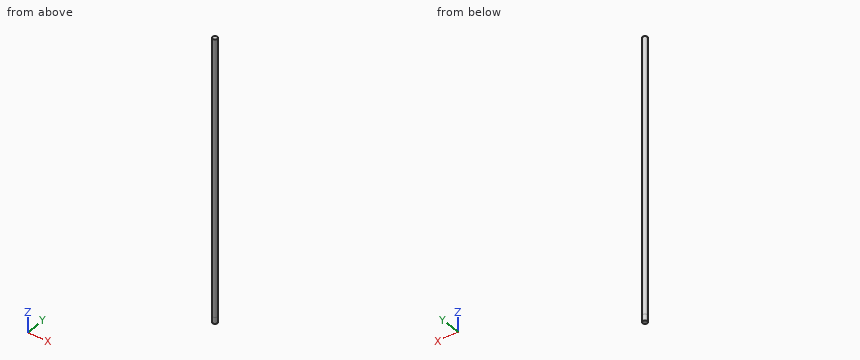
```python
from build123d import *

# Parameters (mm, degrees)
SKETCH_1_R          = 12.5
EXTRUDE_1_DEPTH     = 1470
EXTRUDE_START       = 50
SKETCH_9_R          = 12.5
EXTRUDE_5_DEPTH     = 50
SKETCH_2_W          = 0.55
SKETCH_2_H          = 1.3
CUT_EXTRUDE_START   = -16.5
SKETCH_11_R         = 12.5
CUT_EXTRUDE_2_DEPTH = 16.5
SKETCH_12_R         = 12.5
CUT_EXTRUDE_3_DEPTH = 16.5


with BuildPart() as part:
    # 草图1 → 凸台-拉伸1 (new body)
    with BuildSketch(Plane.XY):
        Circle(SKETCH_1_R)
    extrude(amount=EXTRUDE_1_DEPTH)

    # 草图9 → 凸台-拉伸5 (add)
    with BuildSketch(Plane(origin=(0, 0, 0), x_dir=(-1, 0, 0), z_dir=(0, 0, -1)).offset(EXTRUDE_START)):
        Circle(SKETCH_9_R)
    extrude(amount=-EXTRUDE_5_DEPTH)

    # 草图2 → 切除-旋转1 (revolve, cut)
    with BuildSketch(Plane(origin=(0, 0, 0), x_dir=(1, 0, 0), z_dir=(0, 1, 0)), mode=Mode.PRIVATE) as cut_revolve_1_sk:
        with Locations((12.225, -1450.65)):
            Rectangle(SKETCH_2_W, SKETCH_2_H)
        with Locations((-12.225, -1450.65)):
            Rectangle(SKETCH_2_W, SKETCH_2_H)
        with Locations((-12.225, 30.65)):
            Rectangle(SKETCH_2_W, SKETCH_2_H)
        with Locations((12.225, 30.65)):
            Rectangle(SKETCH_2_W, SKETCH_2_H)
    revolve(cut_revolve_1_sk.sketch.rotate(Axis((0, 0, 1476.033406801), (0, 0, 1)), 180), axis=Axis((0, 0, 1476.033406801), (0, 0, 1)), mode=Mode.SUBTRACT)

    # 草图11 → 切除-拉伸2 (cut)
    with BuildSketch(Plane.XY.offset(1470).offset(CUT_EXTRUDE_START)):
        with Locations(Location((0, 0, 0), (0, 0, 180))):
            Circle(SKETCH_11_R)
    extrude(amount=CUT_EXTRUDE_2_DEPTH, mode=Mode.SUBTRACT)

    # 草图12 → 切除-拉伸3 (cut)
    with BuildSketch(Plane(origin=(0, 0, -50), x_dir=(-1, 0, 0), z_dir=(0, 0, -1))):
        Circle(SKETCH_12_R)
    extrude(amount=-CUT_EXTRUDE_3_DEPTH, mode=Mode.SUBTRACT)


solid = part.part
```
Geometry: final body of the model. Coordinates: model frame, mm. Coordinates: 2 decimals unless noted, no trailing zeros. Order: outer loops, then holes, each group sorted by start corner. A loop starts at its lowest first (then second) coordinate and runs counter-clockwise, first axis right, second up. Notation, with made-up numbers: M 86,-5.75 L 131,-5.75 A29 cw 131,17.25 Z; hole C 79.5,9.5 d1. An arc over 180 degrees is marked long. Answer as CSV lines item,"result".
Q1. Section B-B on x = 6.25. Return the cut outline in (y, z), and give its area (3 significant figures).
Answers:
outline,"M -10.83,-33.5 L 10.83,-33.5 L 10.83,-31.3 L 10.19,-31.3 L 10.19,-30 L 10.83,-30 L 10.83,1450 L 10.19,1450 L 10.19,1451.3 L 10.83,1451.3 L 10.83,1453.5 L -10.83,1453.5 L -10.83,1451.3 L -10.19,1451.3 L -10.19,1450 L -10.83,1450 L -10.83,-30 L -10.19,-30 L -10.19,-31.3 L -10.83,-31.3 Z"
area,"32,200 mm^2"
Q2. Section A-A on y = -7.5. Return the cut outline in (x, z), and give its area (3 significant figures).
Answers:
outline,"M -10,-33.5 L 10,-33.5 L 10,-31.3 L 9.3,-31.3 L 9.3,-30 L 10,-30 L 10,1450 L 9.3,1450 L 9.3,1451.3 L 10,1451.3 L 10,1453.5 L -10,1453.5 L -10,1451.3 L -9.3,1451.3 L -9.3,1450 L -10,1450 L -10,-30 L -9.3,-30 L -9.3,-31.3 L -10,-31.3 Z"
area,"29,700 mm^2"
Q3. Section C-C on z = 643. Return the cut outline in (x, y).
Answers:
outline,"C 0,0 d25"
Q4. Line query: probe 1 along Z at (x, y) = (8, -9.5); probe 2 along X at (y, z) = (3.5, 714); probe 3 along X at (y, z) = (-0.5, 114.5). Output: solid intervals per line, ascending. Write a range as [from, to].
Answers:
probe 1,"z = [-33.5, -31.3], [-30, 1450], [1451.3, 1453.5]"
probe 2,"x = [-12, 12]"
probe 3,"x = [-12.49, 12.49]"
Q5. First-contact query: P1, Ø1.5, axis at x = -5, z = 348, coming from the -Y side; P2, Ø5, axis at y = 9, z = 1293, coming from the -X side. Flat tips, straight axial feed; report the tip coordinate or a pass-through.
Answers:
P1,"stops at y = -11.76"
P2,"stops at x = -10.68"
